Part model, mm, in its own coordinate system. A direction names the side the tool comes from. Coordinates: 2 decimals unless noted, no trailing zeros. Loops run counter-clockwise (first coordinate to the right, second up) from the corner with the lowest first, then second, coordinate; pieces in that order, holes last. Notation, with made-up numbers: (-25.75, 77.5) -> (-8.75, 77.5) arc R9 ccw to (-8.75, 83.5) -> close; hole circle Ø8 at (9.25, -17). An arc over 180 degrees is marked (long way). Use one line per item in the form item = value. Start each with the question number.
(1) Band-saw the part on B-B on z = 0. Give the cut face in (x, y).
(2) Band-saw the part on D-D on x = 24. Give the cut face in (y, z).
(3) Band-saw the part on A-A on y = 16. Give the cut face in (x, z), then the cut area to 3 significant figures.
(4) Drill centre lines: L1, parallel to Z at x = 24, y = 6.25; L2, parallel to Y at x = -8.25, z = 0; L3, parallel to Y at x = 0, z = -1. Where is each one in solid material? Low to high. Write a range as [from, to].
(5) 3-axis set-ups, long thin cutter, end or side, ignore diameter. For faces 1 (the cylindrical face through (-8.42, 17.39, 0.89)), 2 (the flat face through (0, 8, -6)), 3 (the flat face through (11, 13, 0)): which of +Z, -Z, +X, -X, +Y, -Y reach the whole face in a straight line?
(6) Band-saw the part on C-C on z = -3.75. Give the cut face in (x, y), then the cut area to 3 significant figures.
(7) Pin check, flat tips, straight feed: P1, Ø2, axis at x = -6.5, y = 19, coming from the +Z side; P2, Ø6, axis at x = 24, z = 7, coming from the +Y side; P3, Ø11, axis at y = 16.5, z = -0.5, coming from the +X side. Stop position of each tip, or through.
(8) Mould opens along X. For faces 4 (the flat face through (-11, 13, 0)), 5 (the cylindrical face through (10.14, 24.1, -0.07)), 6 (the flat face through (-3, 22, -5)), 7 (the cylindrical face through (-26.146, 4.958, -7.676)) say: +X half, -X half, draft (parallel to the pull), parting line (faces both ways), or undercut.
```python
from build123d import *

# Parameters (mm, degrees)
SKETCH_1_W              = 56
SKETCH_1_H              = 26
EXTRUDE_1_DEPTH         = 8
SKETCH_2_W              = 70.031318806
SKETCH_2_H              = 22.1
CUT_EXTRUDE_1_DEPTH     = 2
SKETCH_3_W              = 22
SKETCH_3_H              = 10
EXTRUDE_2_DEPTH         = 17
SKETCH_4_R              = 6
CUT_EXTRUDE_2_DEPTH     = 46.661800227
HOLE_WIZARD_4_5_4_5_1_D = 4.5
FILLET_2_R              = 3
HOLE_WIZARD_M4_1_D      = 3.3
CHAMFER_1_SIZE          = 1


with BuildPart() as part:
    # 草图1 → 凸台-拉伸1 (new body)
    with BuildSketch(Plane(origin=(0, 0, 0), x_dir=(1, 0, 0), z_dir=(0, 1, 0))):
        Rectangle(SKETCH_1_W, SKETCH_1_H)
    extrude(amount=EXTRUDE_1_DEPTH)

    # 草图2 → 切除-拉伸1 (cut)
    with BuildSketch(Plane.XZ):
        Rectangle(SKETCH_2_W, SKETCH_2_H)
    extrude(amount=-CUT_EXTRUDE_1_DEPTH, mode=Mode.SUBTRACT)

    # 草图3 → 凸台-拉伸2 (add)
    with BuildSketch(Plane(origin=(0, 8, 0), x_dir=(1, 0, 0), z_dir=(0, 1, 0))):
        Rectangle(SKETCH_3_W, SKETCH_3_H)
    extrude(amount=EXTRUDE_2_DEPTH)

    # 草图4 → 切除-拉伸2 (cut, through all)
    with BuildSketch(Plane(origin=(0, 0, -13), x_dir=(-1, 0, 0), z_dir=(0, 0, -1))):
        with Locations((0, 16)):
            Circle(SKETCH_4_R)
    extrude(amount=-CUT_EXTRUDE_2_DEPTH, mode=Mode.SUBTRACT)

    # Ø4.5 (4.5) 直径孔1 (through all)
    with Locations(Plane(origin=(0, 8, 0), x_dir=(1, 0, 0), z_dir=(0, 1, 0))):
        with Locations((-24, 7), (-24, -7), (24, 7), (24, -7)):
            Hole(HOLE_WIZARD_4_5_4_5_1_D / 2)

    # 圆角2
    fillet_2_edges = [part.edges().sort_by_distance(p)[0] for p in [
        (11, 25, 0),
        (-11, 25, 0),
    ]]
    fillet(fillet_2_edges, radius=FILLET_2_R)

    # M4 螺纹孔1 (through all)
    with Locations(Plane(origin=(11, 0, 0), x_dir=(0, 0, -1), z_dir=(1, 0, 0))):
        with Locations((0, 16)):
            Hole(HOLE_WIZARD_M4_1_D / 2)

    # 倒角1
    chamfer_1_edges = [part.edges().sort_by_distance(p)[0] for p in [
        (28, 4, 13),
        (-28, 4, 13),
        (-28, 4, -13),
        (28, 4, -13),
    ]]
    chamfer(chamfer_1_edges, length=CHAMFER_1_SIZE)


solid = part.part
```
A:
q1.outline = (-28, 2) -> (28, 2) -> (28, 8) -> (11, 8) -> (11, 14.35) -> (5.77, 14.35) arc R6 cw to (-5.77, 14.35) -> (-11, 14.35) -> (-11, 8) -> (-28, 8) -> close; (-11, 17.65) -> (-5.77, 17.65) arc R6 cw to (5.77, 17.65) -> (11, 17.65) -> (11, 22) arc R3 ccw to (8, 25) -> (-8, 25) arc R3 ccw to (-11, 22) -> close
q2.outline = (0, -13) -> (8, -13) -> (8, -9.25) -> (2, -9.25) -> (2, -11.05) -> (0, -11.05) -> close; (0, 11.05) -> (2, 11.05) -> (2, 9.25) -> (8, 9.25) -> (8, 13) -> (0, 13) -> close; (2, -4.75) -> (8, -4.75) -> (8, 4.75) -> (2, 4.75) -> close
q3.outline = (-11, -5) -> (-6, -5) -> (-6, -1.65) -> (-11, -1.65) -> close; (-11, 1.65) -> (-6, 1.65) -> (-6, 5) -> (-11, 5) -> close; (6, -5) -> (11, -5) -> (11, -1.65) -> (6, -1.65) -> close; (6, 1.65) -> (11, 1.65) -> (11, 5) -> (6, 5) -> close
q3.area = 67.0 mm²
q4.L1 = [-13, -9.25], [-4.75, 4.75], [9.25, 13]
q4.L2 = [2, 14.35], [17.65, 24.99]
q4.L3 = [2, 10], [22, 25]
q5.face_1 = +X, -X
q5.face_2 = +Y
q5.face_3 = +Z, -Z, +X, +Y
q6.outline = (-28, 2) -> (28, 2) -> (28, 8) -> (11, 8) -> (11, 22) arc R3 ccw to (8, 25) -> (-8, 25) arc R3 ccw to (-11, 22) -> (-11, 8) -> (-28, 8) -> close; hole circle Ø12 at (0, 16)
q6.area = 593 mm²
q7.P1 = 5
q7.P2 = 8
q7.P3 = 11
q8.face_4 = -X half
q8.face_5 = +X half
q8.face_6 = draft
q8.face_7 = undercut
